```python
from build123d import *

# Parameters (mm, degrees)
SKETCH1_R            = 8.25
BOSS_EXTRUDE1_DEPTH  = 3
SKETCH2_R            = 10
BOSS_EXTRUDE2_DEPTH  = 32
SKETCH4_R            = 13
BOSS_EXTRUDE3_DEPTH  = 5
SKETCH5_R            = 7
CUT_EXTRUDE1_DEPTH   = 10
SKETCH6_R            = 2.5
CUT_EXTRUDE2_DEPTH   = 33
SKETCH7_R            = 3.75
CUT_EXTRUDE3_DEPTH   = 6.5
CUT_SWEEP1_PROFILE_R = 2
SKETCH15_W           = 6
SKETCH15_H           = 4.8134745
CUT_EXTRUDE4_START   = -1.5
SKETCH17_R           = 11
SKETCH17_R_2         = 8
CUT_EXTRUDE4_DEPTH   = 1.5


with BuildPart() as part:
    # Sketch1 → Boss-Extrude1 (new body)
    with BuildSketch(Plane(origin=(0, 0, 0), x_dir=(0, 0, -1), z_dir=(1, 0, 0))):
        Circle(SKETCH1_R)
    extrude(amount=BOSS_EXTRUDE1_DEPTH)

    # Sketch2 → Boss-Extrude2 (add)
    with BuildSketch(Plane(origin=(3, 0, 0), x_dir=(0, 0, -1), z_dir=(1, 0, 0))):
        Circle(SKETCH2_R)
    extrude(amount=BOSS_EXTRUDE2_DEPTH)

    # Sketch4 → Boss-Extrude3 (add)
    with BuildSketch(Plane(origin=(35, 0, 0), x_dir=(0, 0, -1), z_dir=(1, 0, 0))):
        Circle(SKETCH4_R)
    extrude(amount=BOSS_EXTRUDE3_DEPTH)

    # Sketch5 → Cut-Extrude1 (cut)
    with BuildSketch(Plane(origin=(40, 0, 0), x_dir=(0, 0, -1), z_dir=(1, 0, 0))):
        Circle(SKETCH5_R)
    extrude(amount=-CUT_EXTRUDE1_DEPTH, mode=Mode.SUBTRACT)

    # Sketch6 → Cut-Extrude2 (cut)
    with BuildSketch(Plane(origin=(30, 0, 0), x_dir=(0, 0, -1), z_dir=(1, 0, 0))):
        Circle(SKETCH6_R)
    extrude(amount=-CUT_EXTRUDE2_DEPTH, mode=Mode.SUBTRACT)

    # Sketch7 → Cut-Extrude3 (cut)
    with BuildSketch(Plane.ZY):
        Circle(SKETCH7_R)
    extrude(amount=-CUT_EXTRUDE3_DEPTH, mode=Mode.SUBTRACT)

    # Cut-Sweep1: sweep along a path in Sketch8
    with BuildLine(Plane.XY) as cut_sweep1_path:
        Line((22, 11.268162534), (22, -10.569361757))
    # Cut-Sweep1 profile (on start of the path) → Cut-Sweep1 (sweep, cut)
    with BuildSketch(Plane(origin=(22, 11.268162534, 0), x_dir=(-1, 0, 0), z_dir=(0, -1, 0))):
        Circle(CUT_SWEEP1_PROFILE_R)
    sweep(path=cut_sweep1_path.line, mode=Mode.SUBTRACT)

    # Sketch15 → Cut-Revolve1 (revolve, cut)
    with BuildSketch(Plane.XY, mode=Mode.PRIVATE) as cut_revolve1_sk:
        with Locations((22, 10.40673725)):
            Rectangle(SKETCH15_W, SKETCH15_H)
    revolve(cut_revolve1_sk.sketch.rotate(Axis((0, 0, 0), (-1, 0, 0)), 90), axis=Axis((0, 0, 0), (-1, 0, 0)), mode=Mode.SUBTRACT)

    # Sketch17 → Cut-Extrude4 (cut)
    with BuildSketch(Plane(origin=(40, 0, 0), x_dir=(0, 0, -1), z_dir=(1, 0, 0)).offset(CUT_EXTRUDE4_START)):
        Circle(SKETCH17_R)
        Circle(SKETCH17_R_2, mode=Mode.SUBTRACT)
    extrude(amount=CUT_EXTRUDE4_DEPTH, mode=Mode.SUBTRACT)


solid = part.part
```
Could you check a few things on this model? Use its own coordinates, in mm. A direction names the side the tool comes from. Round coordinates to 2 decimals unless told otherwise and drop trailing zeros. Order: outer loops, then holes, each group sorted by start corner. A loop starts at its lowest first (then second) coordinate and runs counter-clockwise, first axis right, second up. Notation, with made-up numbers: M 85.5,-1 L 132.5,-1 A19 ccw 132.5,36 Z; hole C -28.5,12.5 d9. An arc over 180 degrees is marked long. One line per question, with ' | ' between items. Start each with the question number.
(1) Please list where these lines run through material, in increasing order: line 1 along X through (y, z) = (5.75, 0); line 2 along Y through (x, z) = (2.75, 0); line 3 along X through (y, z) = (-8.25, 4).
(2) Suppose I cut it at B-B on x = 17. List the corners of the cut face in (y, z) for me, then the cut area to 3 significant figures.
(3) Suppose I cut it at A-A on x = 22.5. List the corners of the cut face in (y, z) for me, then the cut area to 3 significant figures.
(4) For P1, Ø8, axis at x = 27, y = -6.5, coming from the +Z side; P2, Ø6, axis at y = 0, z = 0, coming from the +X side; P3, Ø2.5, axis at x = 22, z = 0, coming from the +Y side; P4, Ø8, axis at x = 8, y = -1, coming from the +Z side, each with a flat end and sliding along its axis, tell me the tip position at first contact or that it passes through.
(5) Suppose I cut it at C-C on z = 0. Count the separate pieces of the cut face and the enclosed holes in it, then the cut area to 3 significant figures.
(6) For faces 5 (the face through (39.24, -10.74, 2.38)), 6 (the face through (6.5, 3, 0)), 7 (the face through (22, 5, 2)), which set-ups out of +Z, -Z, +X, -X, +Y, -Y let a thin tool reach every point of the face, with its end or its side?
(7) Thinking about a two-plate mould opening in X: for faces 1 (the face through (0, -4, -2)), 2 (the face through (19, -8.2, 0)), 3 (the face through (25, -8.2, 0)), 4 (the face through (29.93, -9.76, 2.17)), which applies, +X half, -X half, draft (parallel to the pull), parting line (faces both ways), or undercut?
Geometry results:
1) line 1: 0 to 20, 24 to 30 | line 2: -8.25 to -3.75, 3.75 to 8.25 | line 3: 3 to 19, 25 to 38.5
2) outline: C 0,0 d20; hole C 0,0 d5 | area: 295 mm²
3) outline: M -7.76,-1.94 A8 ccw 7.76,-1.94 L 1.58,-1.94 A2.5 cw -1.58,-1.94 Z; M -7.76,1.94 L -1.58,1.94 A2.5 cw 1.58,1.94 L 7.76,1.94 A8 ccw Z | area: 137 mm²
4) P1: z = 9.68 | P2: x = 30 | P3: through | P4: z = 10
5) separate pieces: 4 | enclosed holes: 0 | area: 436 mm²
6) face 5: +X | face 6: -X | face 7: +Y, -Y
7) face 1: -X half | face 2: undercut | face 3: undercut | face 4: draft
